from build123d import *

# Parameters (mm, degrees)
CUT_EXTRUDE1_DEPTH = 2
CHAMFER1_SIZE      = 0.5


with BuildPart() as part:
    # Sketch1 → Revolve1 (revolve)
    with BuildSketch(Plane.XY, mode=Mode.PRIVATE) as revolve1_sk:
        Polygon((0, 0), (0, 25.5), (-4.5, 25.5), (-4.5, 22), (-2.5, 22), (-2.5, 8), (-2, 8), (-2, 0), align=None)
    revolve(revolve1_sk.sketch.rotate(Axis((0, 0, 0), (0, 1, 0)), 180), axis=Axis((0, 0, 0), (0, 1, 0)))

    # Sketch2 → Cut-Extrude1 (cut)
    with BuildSketch(Plane(origin=(0, 25.5, 0), x_dir=(1, 0, 0), z_dir=(0, 1, 0))):
        Polygon((1.554085232, -0.764734655), (1.439322254, 0.963509963), (-0.114762978, 1.728244618), (-1.554085232, 0.764734655), (-1.439322254, -0.963509963), (0.114762978, -1.728244618), align=None)
    extrude(amount=-CUT_EXTRUDE1_DEPTH, mode=Mode.SUBTRACT)

    # Chamfer1
    chamfer1_edges = [part.edges().sort_by_distance(p)[0] for p in [
        (-4.5, 22, 0),
        (-4.5, 25.5, 0),
    ]]
    chamfer(chamfer1_edges, length=CHAMFER1_SIZE)


solid = part.part
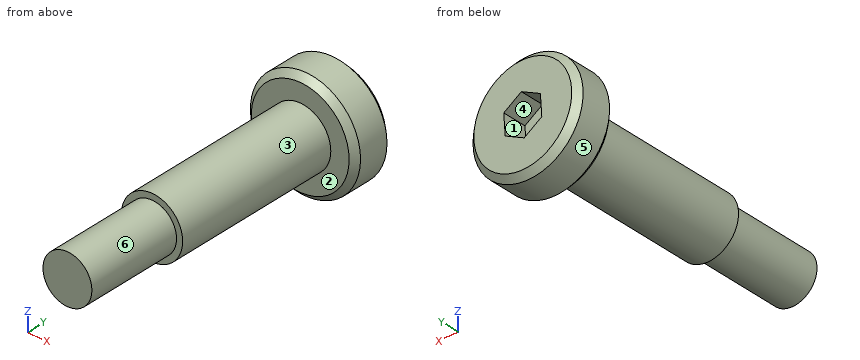
The model under review builds one solid part; all positions refer to its coordinate system, in mm. Face numbers are marked on the shaded views. A direction names the side the tool comes from. Give positions to 0.01 mm unless a question says otherwise; leave off trailing zeros. Order: outer loops, then holes, each group sorted by start corner. A loop starts at its lowest first (then second) coordinate and runs counter-clockwise, first axis right, second up. Notation, with made-up numbers: M -16.75,-31.75 L 34.25,-31.75 A6 cw 34.25,-26.75 Z; hole C 60.5,-11 d10. An arc over 180 degrees is marked long. Answer in a Markdown table with one row per item. Add a question column.
1. Machinability: for the marked faces 4, 5 and 6, which of the approach directions +Z, -Z, +X, -X, +Y, -Y give a long, thin tool a straight path to every point of the face, cutting with its end or side? Answer none if there is none.
2. Add section A-A on y = 23.75. State the section outline as (x, z) points, plus the area to 3 significant figures.
3. Add section B-B on y = 9.5. State the section outline as (x, z) points.
4. For pin 1 Ø4 at (x, z) = (0.5, 0.5) entering from -Y; pin 2 Ø4 at (y, z) = (19, 0.5) entering from -X; pin 3 Ø1.5 at (y, z) = (11, -2) entering from +X; pin 4 Ø1 at (y, z) = (17.5, -2) entering from +X, all flat-tipped, find the tip position at first contact; note any pin that passes through.
5. Mouldability with a two-part tool opening along Z and no side actions: class the marked faces 1, 2 and 3 as released by +Z, released by -Z, zero draft, split by the parting line, or undercut.
6. To check wall thickness, follow line 1 along Y through (x, z) = (-0.25, 1); line 2 along Y through (x, z) = (-0.25, -3.5); line 3 along X through (y, z) = (24.25, -0.75). State the ranges of each line that lie inside material, in increasing order.
The answers:
| question | item | result |
|---|---|---|
| 1 | face 4 | +Y |
| 1 | face 5 | +Y, -Y |
| 1 | face 6 | -Y |
| 2 | outline | C 0,0 d9; hole M -1.55,-0.76 L -0.11,-1.73 L 1.44,-0.96 L 1.55,0.76 L 0.11,1.73 L -1.44,0.96 Z |
| 2 | area | 55.8 mm2 |
| 3 | outline | C 0,0 d5 |
| 4 | pin 1 | y = 0 |
| 4 | pin 2 | x = -2.5 |
| 4 | pin 3 | x = 2.17 |
| 4 | pin 4 | x = 2 |
| 5 | face 1 | undercut |
| 5 | face 2 | zero draft |
| 5 | face 3 | split by the parting line |
| 6 | line 1 | 0 to 23.5 |
| 6 | line 2 | 22 to 25.5 |
| 6 | line 3 | -4.44 to -1.55, 1.45 to 4.44 |
